Build history of the part. All positions in model axes, mm. A direction names the side the tool comes from. Coordinates: 2 decimals unless noted, no trailing zeros. Order: outer loops, then holes, each group sorted by start corner. A loop starts at its lowest first (then second) coordinate and runs counter-clockwise, first axis right, second up. Notation, with made-up numbers: M 54.25,60 L 63.25,60 A20 cw 63.25,74 Z; hole C 35,-37.75 d5. An arc over 180 degrees is marked long. Use a Markdown table: item, result. Add a question column.
from build123d import *

# Parameters (mm, degrees)
CHAMFER1_SIZE = 0.5


with BuildPart() as part:
    # Sketch1 → Revolve1 (revolve)
    with BuildSketch(Plane(origin=(0, 0, 0), x_dir=(0, 0, -1), z_dir=(1, 0, 0)), mode=Mode.PRIVATE) as revolve1_sk:
        Polygon((11, 0), (11, 7.5), (8, 7.5), (8, 5), (0, 5), (0, 0), align=None)
    revolve(revolve1_sk.sketch.rotate(Axis((0, 0, 0), (0, 0, -1)), 90), axis=Axis((0, 0, 0), (0, 0, -1)))

    # Chamfer1
    chamfer1_edges = [part.edges().sort_by_distance(p)[0] for p in [
        (-5, 0, 0),
        (-7.5, 0, -8),
        (-7.5, 0, -11),
    ]]
    chamfer(chamfer1_edges, length=CHAMFER1_SIZE)


solid = part.part
(1) Slice it at D-D on z = -9. Give the cut face in (x, y), and give its area (3 significant figures).
(2) Slice it at C-C on z = -2.25. Give the cut face in (x, y).
(3) Slice it at A-A on x = 0. Give the cut face in (y, z).
(4) Drill centre lines: line 1 along X through (y, z) = (0.25, -9); line 2 along Z through (x, y) = (5, -2); line 3 along X through (y, z) = (2.5, -0.25). Where is each one in solid material? Low to high. Write a range as from..to.
(5) Which spindle directions (+Z, -Z, +X, -X, +Y, -Y) get a long thin tool onto all of the face, cutting with end or side? Do faces 1 (the cylindrical face through (-5, 0, -4)), 2 (the flat face through (0, 0, -11)). Say none if no direction does.
(6) Drop flat-ended pins along their axis: P1, Ø2, axis at y = 1.5, z = -3, coming from the +X side; P2, Ø7, axis at x = -2.5, y = 3, coming from the +Z side; P3, Ø2, axis at x = 2, z = -9, coming from the +Y side; P4, Ø2, axis at x = 1, y = -5.5, coming from the +Z side. Give the stop position or say it passes through.
Solutions:
| question | item | result |
|---|---|---|
| 1 | outline | C 0,0 d15 |
| 1 | area | 177 mm² |
| 2 | outline | C 0,0 d10 |
| 3 | outline | M -7.5,-10.5 L -7,-11 L 7,-11 L 7.5,-10.5 L 7.5,-8.5 L 7,-8 L 5,-8 L 5,-0.5 L 4.5,0 L -4.5,0 L -5,-0.5 L -5,-8 L -7,-8 L -7.5,-8.5 Z |
| 4 | line 1 | -7.5..7.5 |
| 4 | line 2 | -11..-8 |
| 4 | line 3 | -4.04..4.04 |
| 5 | face 1 | +Z |
| 5 | face 2 | -Z, +X, -X, +Y, -Y |
| 6 | P1 | x = 4.97 |
| 6 | P2 | z = 0 |
| 6 | P3 | y = 7.43 |
| 6 | P4 | z = -0.09 |
